```python
from build123d import *

# Parameters (mm, degrees)
BOSS_EXTRUDE1_DEPTH                                  = 67.5
M8_TAPPED_HOLE1_D                                    = 6.8
M8_TAPPED_HOLE1_DEPTH                                = 19.75
M8_TAPPED_HOLE1_TIP                                  = 2.042926105
HOLE_SIZE_PER_SOCKET_HEAD_CAP_SCREW_TYPE_D           = 11
HOLE_SIZE_PER_SOCKET_HEAD_CAP_SCREW_TYPE_CBORE_D     = 18
HOLE_SIZE_PER_SOCKET_HEAD_CAP_SCREW_TYPE_CBORE_DEPTH = 11
SKETCH8_R                                            = 21
CUT_EXTRUDE1_DEPTH                                   = 260.723410574
M8_TAPPED_HOLE2_D                                    = 6.8
M8_TAPPED_HOLE2_DEPTH                                = 19.75
M8_TAPPED_HOLE2_TIP                                  = 2.042926105
CHAMFER1_SIZE                                        = 2
M3_TAPPED_HOLE1_D                                    = 2.5
M3_TAPPED_HOLE1_DEPTH                                = 7.5
M3_TAPPED_HOLE1_TIP                                  = 0.751075774


with BuildPart() as part:
    # Sketch1 → Boss-Extrude1 (new, symmetric)
    with BuildSketch(Plane.XY):
        Polygon((0, 0), (0, 60), (10, 80), (10, 250), (30, 250), (30, 0), align=None)
    extrude(amount=BOSS_EXTRUDE1_DEPTH, both=True)

    # M8 Tapped Hole1
    with Locations(Plane.XZ):
        with Locations((6, -42.5), (24, -42.5), (24, 0), (6, 0), (6, 42.5), (24, 42.5)):
            Hole(M8_TAPPED_HOLE1_D / 2, depth=M8_TAPPED_HOLE1_DEPTH)
            with Locations((0, 0, -(M8_TAPPED_HOLE1_DEPTH + M8_TAPPED_HOLE1_TIP / 2))):  # 118° drill point
                Cone(0, M8_TAPPED_HOLE1_D / 2, M8_TAPPED_HOLE1_TIP, mode=Mode.SUBTRACT)

    # Hole size per socket head cap screw type1 (through all)
    with Locations(Plane(origin=(30, 0, 0), x_dir=(0, 0, -1), z_dir=(1, 0, 0))):
        with Locations((-40, 232.5), (40, 232.5), (40, 92.5), (-40, 92.5), (0, 232.5), (0, 92.5)):
            CounterBoreHole(HOLE_SIZE_PER_SOCKET_HEAD_CAP_SCREW_TYPE_D / 2, HOLE_SIZE_PER_SOCKET_HEAD_CAP_SCREW_TYPE_CBORE_D / 2, HOLE_SIZE_PER_SOCKET_HEAD_CAP_SCREW_TYPE_CBORE_DEPTH)

    # Sketch8 → Cut-Extrude1 (cut, through all)
    with BuildSketch(Plane.ZY.offset(-10)):
        with Locations(Location((0, 162.5, 0), (0, 0, 270))):
            Circle(SKETCH8_R)
    extrude(amount=-CUT_EXTRUDE1_DEPTH, mode=Mode.SUBTRACT)

    # M8 Tapped Hole2
    with Locations(Plane(origin=(0, 250, 0), x_dir=(-1, 0, 0), z_dir=(0, 1, 0))):
        with Locations((-20, -25), (-20, 25)):
            Hole(M8_TAPPED_HOLE2_D / 2, depth=M8_TAPPED_HOLE2_DEPTH)
            with Locations((0, 0, -(M8_TAPPED_HOLE2_DEPTH + M8_TAPPED_HOLE2_TIP / 2))):  # 118° drill point
                Cone(0, M8_TAPPED_HOLE2_D / 2, M8_TAPPED_HOLE2_TIP, mode=Mode.SUBTRACT)

    # Chamfer1
    chamfer1_edges = [part.edges().sort_by_distance(p)[0] for p in [
        (20, 250, 67.5),
        (20, 250, -67.5),
    ]]
    chamfer(chamfer1_edges, length=CHAMFER1_SIZE)

    # M3 Tapped Hole1
    with Locations(Plane.ZY.offset(-10)):
        with Locations((-37.5, 152.5), (-37.5, 172.5)):
            Hole(M3_TAPPED_HOLE1_D / 2, depth=M3_TAPPED_HOLE1_DEPTH)
            with Locations((0, 0, -(M3_TAPPED_HOLE1_DEPTH + M3_TAPPED_HOLE1_TIP / 2))):  # 118° drill point
                Cone(0, M3_TAPPED_HOLE1_D / 2, M3_TAPPED_HOLE1_TIP, mode=Mode.SUBTRACT)


solid = part.part
```
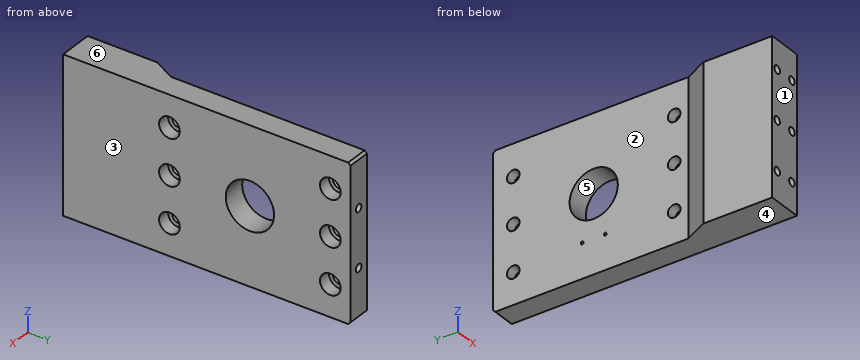
Geometry: final body of the model. Coordinates: model frame, mm. Face numbers are marked on the shaded views. A direction names the side the tool comes from. Give positions to 0.01 mm unless a question says otherwise; leave off trailing zeros. Loops run counter-clockwise (first coordinate to the right, second up) from the corner with the lowest first, then second, coordinate; pieces in that order, holes last. Notation, with made-up numbers: (25, 64) -> (39, 64) arc R8 ccw to (39, 72) -> close; hole circle Ø9 at (10, -10.5). An arc over 180 degrees is marked (long way). Use one line per item in the form item = value.
Item 1: Section query A-A on y = 162.5. Output: boundary loops of the cut face in (x, z).
A:
outline = (10, -67.5) -> (30, -67.5) -> (30, -21) -> (10, -21) -> close; (10, 21) -> (30, 21) -> (30, 67.5) -> (10, 67.5) -> close
Item 2: Draft query along Z for the marked faces 3, 4, 5 and 6. Return one class per face: pulls with the +Z half, pulls with the -Z half, needs draft (parallel to the pull), parting line crosses it, or undercut.
A:
face_3 = needs draft
face_4 = pulls with the -Z half
face_5 = undercut
face_6 = pulls with the +Z half
Item 3: Section query B-B on x = 13. Give the number of separate pieces and of enclosed holes in the cut face, and give its area (3 significant figures).
A:
separate_pieces = 1
enclosed_holes = 9
area = 31,800 mm^2
Item 4: Section query C-C on y = 92.5. Output: boundary loops of the cut face in (x, z).
A:
outline = (10, -67.5) -> (30, -67.5) -> (30, -49) -> (19, -49) -> (19, -45.5) -> (10, -45.5) -> close; (10, -34.5) -> (19, -34.5) -> (19, -31) -> (30, -31) -> (30, -9) -> (19, -9) -> (19, -5.5) -> (10, -5.5) -> close; (10, 5.5) -> (19, 5.5) -> (19, 9) -> (30, 9) -> (30, 31) -> (19, 31) -> (19, 34.5) -> (10, 34.5) -> close; (10, 45.5) -> (19, 45.5) -> (19, 49) -> (30, 49) -> (30, 67.5) -> (10, 67.5) -> close
Item 5: Pin query (flat end, axial travel): P1, Ø8, axis at y = 149.5, z = -42, coming from the -X side; P2, Ø3, axis at x = 5, z = -5, coming from the +Y side; P3, Ø9, axis at x = 6, z = 0, coming from the +Y side; P4, Ø2, axis at x = 3.5, z = 7, coming from the +Y side. Return the tip coordinate at first contact, or that it passes through.
A:
P1 = 10
P2 = 73
P3 = 250
P4 = 69
Item 6: Section query D-D on z = 58. Output: boundary loops of the cut face in (x, y).
A:
outline = (0, 0) -> (30, 0) -> (30, 250) -> (10, 250) -> (10, 80) -> (0, 60) -> close
Item 7: Line query: probe 1 along Z at (x, y) = (6, 12.75); probe 2 along Y at (x, z) = (21.5, -40); probe 3 along Y at (x, z) = (26.75, 7.5). Output: solid intervals per line, ascending.
A:
probe_1 = -67.5 to -45.9, -39.1 to -3.4, 3.4 to 39.1, 45.9 to 67.5
probe_2 = 0 to 83.5, 101.5 to 223.5, 241.5 to 250
probe_3 = 0 to 87.53, 97.47 to 142.88, 182.12 to 227.53, 237.47 to 250
Item 8: Access query for the marked faces 1 and 2. Directions: +Z, -Z, +X, -X, +Y, -Y. A direction counts if a zero-diameter tool reaches every point of the face in a straight line with its end or side. Return the directions, or none.
A:
face_1 = +Z, -Z, +X, -X, -Y
face_2 = +Z, -Z, -X, +Y
